Source: CAD feature listing. Evaluate the final solid. Frame: model axes, mm. A direction names the side the tool comes from. Give positions to 0.01 mm unless a question says otherwise; leave off trailing zeros. Order: outer loops, then holes, each group sorted by start corner. A loop starts at its lowest first (then second) coordinate and runs counter-clockwise, first axis right, second up. Notation, with made-up numbers: (-8.75, 8.25) -> (9.25, 8.25) arc R34 cw to (9.25, 40.25) -> close; hole circle Ø2 at (58.25, 23.25). An arc over 180 degrees is marked (long way). Use one line per item in the form item = value. Start each with the question number.
from build123d import *

# Parameters (mm, degrees)
SKETCH_1_W                = 105
SKETCH_1_H                = 40
EXTRUDE_1_DEPTH           = 18
SKETCH_2_W                = 30
SKETCH_2_H                = 40
CUT_EXTRUDE_1_DEPTH       = 5
SKETCH_3_W                = 60
SKETCH_3_H                = 40
CUT_EXTRUDE_2_DEPTH       = 8
HOLE_WIZARD_1_D           = 6.6
HOLE_WIZARD_1_CBORE_D     = 11
HOLE_WIZARD_1_CBORE_DEPTH = 6.8
SKETCH_6_R                = 5
CUT_EXTRUDE_3_DEPTH       = 2
CHAMFER_1_SIZE            = 3
CUT_EXTRUDE_4_DEPTH       = 59.993643725
HOLE_WIZARD_M6_1_REACH    = 110.393
HOLE_WIZARD_M6_1_BORE_R   = 3.3
HOLE_WIZARD_M5_1_D        = 4.2


with BuildPart() as part:
    # 草图1 → 凸台-拉伸1 (new body)
    with BuildSketch(Plane.XY):
        Rectangle(SKETCH_1_W, SKETCH_1_H)
    extrude(amount=EXTRUDE_1_DEPTH)

    # 草图2 → 切除-拉伸1 (cut)
    with BuildSketch(Plane(origin=(0, 0, 0), x_dir=(-1, 0, 0), z_dir=(0, 0, -1))):
        with Locations((37.5, 0)):
            Rectangle(SKETCH_2_W, SKETCH_2_H)
    extrude(amount=-CUT_EXTRUDE_1_DEPTH, mode=Mode.SUBTRACT)

    # 草图3 → 切除-拉伸2 (cut)
    with BuildSketch(Plane(origin=(0, 0, 0), x_dir=(-1, 0, 0), z_dir=(0, 0, -1))):
        with Locations((-22.5, 0)):
            Rectangle(SKETCH_3_W, SKETCH_3_H)
    extrude(amount=-CUT_EXTRUDE_2_DEPTH, mode=Mode.SUBTRACT)

    # 打孔尺寸(%根据)内六角圆柱头螺钉的类型1 (through all)
    with Locations(Plane.XY.offset(18)):
        with Locations((-46, 0), (-30.5, 0), (-15, 0)):
            CounterBoreHole(HOLE_WIZARD_1_D / 2, HOLE_WIZARD_1_CBORE_D / 2, HOLE_WIZARD_1_CBORE_DEPTH)

    # 草图6 → 切除-拉伸3 (cut)
    with BuildSketch(Plane(origin=(0, 0, 0), x_dir=(-1, 0, 0), z_dir=(0, 0, -1))):
        with Locations((15, 0)):
            Circle(SKETCH_6_R)
    extrude(amount=-CUT_EXTRUDE_3_DEPTH, mode=Mode.SUBTRACT)

    # 倒角1
    chamfer_1_edges = [part.edges().sort_by_distance(p)[0] for p in [
        (-22.5, -20, 2.5),
        (-22.5, 20, 2.5),
        (-7.5, 20, 4),
        (-7.5, -20, 4),
        (52.5, -20, 13),
        (-52.5, -20, 11.5),
        (-52.5, 20, 11.5),
        (52.5, 20, 13),
    ]]
    chamfer(chamfer_1_edges, length=CHAMFER_1_SIZE)

    # 草图7 → 切除-拉伸4 (cut, through all)
    with BuildSketch(Plane.XY.offset(18)):
        with BuildLine():
            Line((7.5, 5), (37.5, 5))
            ThreePointArc((37.5, 5), (42.5, 0), (37.5, -5))
            Line((37.5, -5), (7.5, -5))
            ThreePointArc((7.5, -5), (2.5, 0), (7.5, 5))
        make_face()
    extrude(amount=-CUT_EXTRUDE_4_DEPTH, mode=Mode.SUBTRACT)

    # M6 间隙孔1 bore → M6 间隙孔1 (cut, up to next)
    with BuildSketch(Plane(origin=(52.5, 0, 0), x_dir=(0, 0, -1), z_dir=(1, 0, 0)), mode=Mode.PRIVATE) as hole_wizard_m6_1_sk1:
        with Locations((-13, 0)):
            Circle(HOLE_WIZARD_M6_1_BORE_R)
    hole_wizard_m6_1_tool1 = extrude(hole_wizard_m6_1_sk1.sketch, amount=-HOLE_WIZARD_M6_1_REACH, mode=Mode.PRIVATE) & part.part
    add(hole_wizard_m6_1_tool1.solids().sort_by_distance((52.5, 0, 13))[0], mode=Mode.SUBTRACT)

    # M5 螺纹孔1 (through all)
    with Locations(Plane.XY.offset(18)):
        with Locations((-2.5, 7.5), (-2.5, -7.5)):
            Hole(HOLE_WIZARD_M5_1_D / 2)


solid = part.part
1) Cut plane B-B, the plane z = 13. Return the cut outline in (x, y), plus the area to 3 significant figures.
2) Reachability of faces 4 (the face through (-42, 0, 11.2)), 5 (the face through (41.259, 3.297, 14.181)), 6 (the face through (-9, 18.5, 3.9)), 7 (the face through (-22.5, 0, 2)), 8 (the face through (46.96, -1.26, 9.95)) from +Z, -Z, +X, -X, +Y, -Y: full face, straight path, thin tool, end or side. Return the list, or none.
3) Draft query along X for faces 1 (the face through (-51, 18.5, 11.4)), 2 (the face through (-42.7, 0.1, 8.1)), 3 (the face through (-7.5, 0, 4)). Return one class per face: +X half, -X half, draft (parallel to the pull), parting line (faces both ways), or undercut.
4) Material intervals for probe 1 along Y at (x, z) = (48, 13); probe 2 along Y at (x, z) = (-46, 15); probe 3 along Z at (x, y) = (-36.5, 3.5), sorted ascending.
5) Cut plane D-D, the plane y = 7.5. Return the cut outline in (x, z).
6) Cut plane A-A, the plane x = -15. Return the cut outline in (y, z), plus the area to 3 significant figures.
7) Pin query (flat end, axial travel): pin 1 (3 mm diameter, centred on x = 14.5, z = 5, fed in from -Y); pin 2 (10.5 mm diameter, centred on x = -15, y = 0, fed in from -Z); pin 3 (5.5 mm diameter, centred on x = -29, y = -2, fed in from +Z); pin 4 (4 mm diameter, centred on y = 4.5, z = 3.5, fed in from +X). Return the tip coordinate at first contact, or that it passes through.
8) Cut plane C-C, the plane x = -2.5. Return the cut outline in (y, z), plus the area to 3 significant figures.
Output values:
q1.outline = (-52.5, -17) -> (-49.5, -20) -> (49.5, -20) -> (52.5, -17) -> (52.5, -3.3) -> (41.26, -3.3) arc R5 cw to (37.5, -5) -> (7.5, -5) arc R5 cw to (7.5, 5) -> (37.5, 5) arc R5 cw to (41.26, 3.3) -> (52.5, 3.3) -> (52.5, 17) -> (49.5, 20) -> (-49.5, 20) -> (-52.5, 17) -> close; hole circle Ø11 at (-46, 0); hole circle Ø11 at (-30.5, 0); hole circle Ø11 at (-15, 0); hole circle Ø4.2 at (-2.5, -7.5); hole circle Ø4.2 at (-2.5, 7.5)
q1.area = 3,420 mm^2
q2.face_4 = +Z
q2.face_5 = +Z, -Z
q2.face_6 = -Z, +X, +Y
q2.face_7 = -Z, -X, +Y, -Y
q2.face_8 = +X
q3.face_1 = -X half
q3.face_2 = undercut
q3.face_3 = +X half
q4.probe_1 = -20 to -3.3, 3.3 to 20
q4.probe_2 = -20 to -5.5, 5.5 to 20
q4.probe_3 = 5 to 18
q5.outline = (-52.5, 5) -> (-22.5, 5) -> (-22.5, 0) -> (-7.5, 0) -> (-7.5, 8) -> (-4.6, 8) -> (-4.6, 18) -> (-52.5, 18) -> close; (-0.4, 8) -> (52.5, 8) -> (52.5, 18) -> (-0.4, 18) -> close
q6.outline = (-20, 0) -> (-5, 0) -> (-5, 2) -> (-3.3, 2) -> (-3.3, 11.2) -> (-5.5, 11.2) -> (-5.5, 18) -> (-20, 18) -> close; (3.3, 2) -> (5, 2) -> (5, 0) -> (20, 0) -> (20, 18) -> (5.5, 18) -> (5.5, 11.2) -> (3.3, 11.2) -> close
q6.area = 564 mm^2
q7.pin_1 = through
q7.pin_2 = 0
q7.pin_3 = 11.2
q7.pin_4 = -7.5
q8.outline = (-20, 8) -> (-9.6, 8) -> (-9.6, 18) -> (-20, 18) -> close; (-5.4, 8) -> (5.4, 8) -> (5.4, 18) -> (-5.4, 18) -> close; (9.6, 8) -> (20, 8) -> (20, 18) -> (9.6, 18) -> close
q8.area = 316 mm^2
